```python
from build123d import *

# Parameters (mm, degrees)
SKETCH_1_R             = 12.5
EXTRUDE_1_DEPTH        = 280
HOLE_WIZARD_M8_1_D     = 6.8
HOLE_WIZARD_M8_1_DEPTH = 22.25
HOLE_WIZARD_M8_1_TIP   = 2.042926105
HOLE_WIZARD_M8_2_D     = 6.8
HOLE_WIZARD_M8_2_DEPTH = 22.25
HOLE_WIZARD_M8_2_TIP   = 2.042926105
CHAMFER_1_SIZE         = 0.5


with BuildPart() as part:
    # 草图1 → 凸台-拉伸1 (new body)
    with BuildSketch(Plane.XY):
        Circle(SKETCH_1_R)
    extrude(amount=EXTRUDE_1_DEPTH)

    # M8 螺纹孔1
    with Locations(Plane.XY.offset(280)):
        with Locations((0, 0)):
            Hole(HOLE_WIZARD_M8_1_D / 2, depth=HOLE_WIZARD_M8_1_DEPTH)
            with Locations((0, 0, -(HOLE_WIZARD_M8_1_DEPTH + HOLE_WIZARD_M8_1_TIP / 2))):  # 118° drill point
                Cone(0, HOLE_WIZARD_M8_1_D / 2, HOLE_WIZARD_M8_1_TIP, mode=Mode.SUBTRACT)

    # M8 螺纹孔2
    with Locations(Plane(origin=(0, 0, 0), x_dir=(-1, 0, 0), z_dir=(0, 0, -1))):
        with Locations((0, 0)):
            Hole(HOLE_WIZARD_M8_2_D / 2, depth=HOLE_WIZARD_M8_2_DEPTH)
            with Locations((0, 0, -(HOLE_WIZARD_M8_2_DEPTH + HOLE_WIZARD_M8_2_TIP / 2))):  # 118° drill point
                Cone(0, HOLE_WIZARD_M8_2_D / 2, HOLE_WIZARD_M8_2_TIP, mode=Mode.SUBTRACT)

    # 倒角1
    chamfer_1_edges = [part.edges().sort_by_distance(p)[0] for p in [
        (-12.5, 0, 0),
        (-12.5, 0, 280),
    ]]
    chamfer(chamfer_1_edges, length=CHAMFER_1_SIZE)


solid = part.part
```
Model file for the job. Use its own axes, mm. A direction names the side the tool comes from. Coordinates: 2 decimals unless noted, no trailing zeros. Loops run counter-clockwise (first coordinate to the right, second up) from the corner with the lowest first, then second, coordinate; pieces in that order, holes last. Notation, with made-up numbers: (62.5, 35) -> (78.5, 35) arc R22 cw to (78.5, 66) -> close; hole circle Ø9 at (67, -8.75). An arc over 180 degrees is marked (long way). Answer as a JSON object with one key per item and string values.
Q1. 3-axis set-ups, long thin cutter, end or side, ignore diameter. For faces 5 (the cylindrical face through (-0.74, -3.32, 11.28)), 6 (the flat face through (2, 3, 280)), 7 (the cylindrical face through (0.74, -3.32, 268.72)): which of +Z, -Z, +X, -X, +Y, -Y reach the whole face in a straight line?
Report:
{"face 5": "-Z", "face 6": "+Z, +X, -X, +Y, -Y", "face 7": "+Z"}
Q2. Pull direction Y, two halves, no side cores. Call faces 1 (the conical face through (0.128, -0.576, 23.938)), 2 (the flat face through (2, 3, 0)), 3 (the cylindrical face through (11.923, 3.755, 138.047)), 4 (the conical face through (-0.128, -0.576, 256.062)): released by +Y, released by -Y, zero draft, split by the parting line, or undercut.
Report:
{"face 1": "undercut", "face 2": "zero draft", "face 3": "split by the parting line", "face 4": "undercut"}
Q3. Probe probe 1 along Y at (x, z) = (0, 14); probe 2 along X at (y, z) = (-1, 254); probe 3 along X at (y, z) = (2.5, 63). List the from-to ranges inside material, lowest first.
Report:
{"probe 1": "y = -12.5 to -3.4, 3.4 to 12.5", "probe 2": "x = -12.46 to 12.46", "probe 3": "x = -12.25 to 12.25"}
Q4. Cut at A-A (z = 68.5). List the corners of the cut face in (x, y).
Report:
{"outline": "circle Ø25 at (0, 0)"}
Q5. Flat gauge pins, fed straight in: P1, Ø5.5, axis at x = 0, y = 0, coming from the -Z side; P2, Ø8, axis at x = 6.5, z = 159, coming from the +Y side; P3, Ø6, axis at y = -4, z = 45, coming from the -X side. Where does each tip first touch, or does it go through?
Report:
{"P1": "stops at z = 22.64", "P2": "stops at y = 12.25", "P3": "stops at x = -12.46"}
